Study the drawing (mm; zero at the part's minimum x, y, z) and answer. A direction names the side the tool comes from. Coordinates: 2 decimals unless noted, no trailing zeros. Write each loop counter-clockwise with the first axis right and the second up, starting at its lowest first coordinate (ties: lowest second). Pieces come first, ordered by that corner, then holes. Notation, with made-up numbers: (9, 24.5) - (60, 24.5) arc R13 ccw to (60, 47.5) - close; hole circle Ø10 at (1.25, 40). An arc over 180 degrees is marked (long way). One line per item, written item: value.
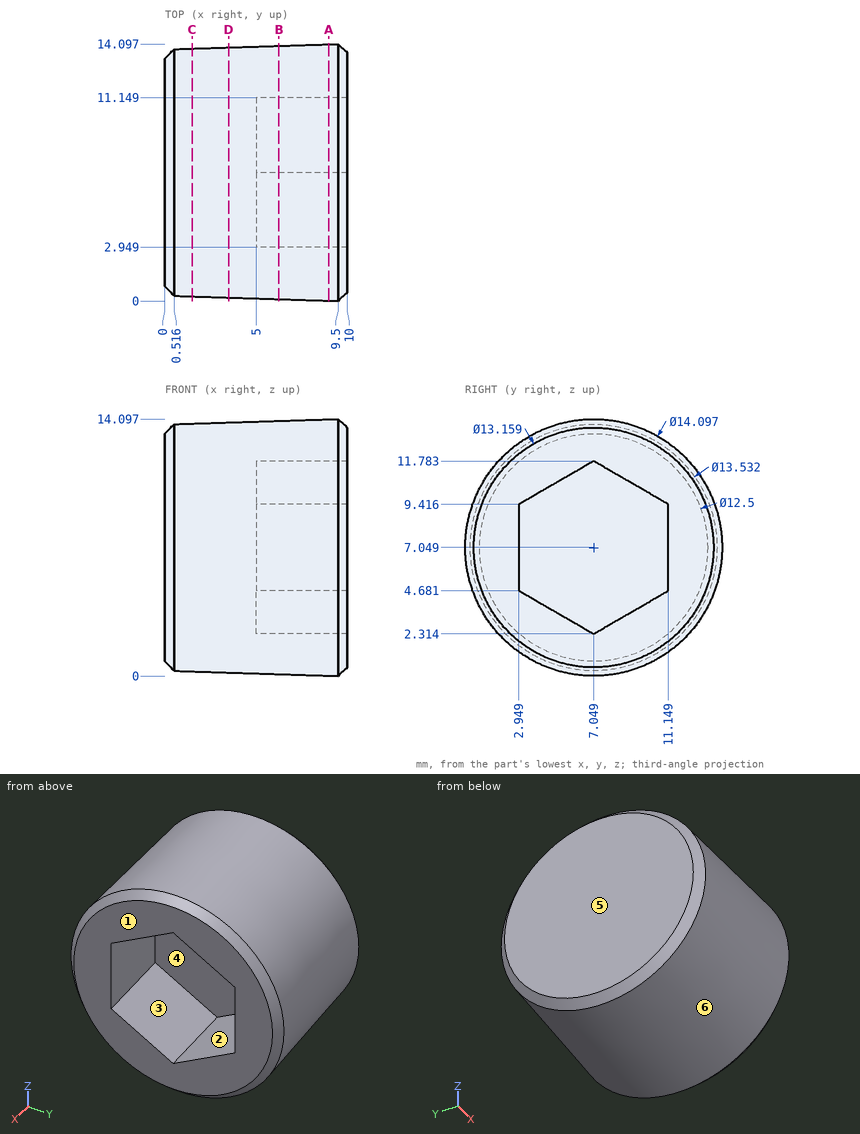
Item 1: Determine the mould class of the marked faces 3, 4, 5 and 6 for opening direction Y: +Y half, -Y half, draft (parallel to the pull), parting line (faces both ways), or undercut.
Evaluation:
face 3: undercut
face 4: undercut
face 5: draft
face 6: parting line
Item 2: Section C-C, the plane x = 1.5 is taken. Determine the outline of the cut face in (y, z) (1 decimal), then the cut area to 3 significant figures.
Evaluation:
outline: circle Ø13.6 at (7, 7)
area: 145 mm2
Item 3: Given pin 1 (6 mm diameter, centred on x = 2, z = 7, fed in from +Y); pin 2 (2 mm diameter, centred on y = 7, z = 4, fed in from -X); pin 3 (2.5 mm diameter, centred on y = 7, z = 7, fed in from +X); pin 4 (6 mm diameter, centred on x = 2, z = 12.5, fed in from -Y), each flat-ended and moving along its own axis, determine where each tip first touches the part or whether it passes through.
Evaluation:
pin 1: stops at y = 13.96
pin 2: stops at x = 0
pin 3: stops at x = 5
pin 4: stops at y = 0.69
Item 4: Section A-A, the plane x = 9 is taken. Determine the outline of the cut face in (y, z) (1 decimal).
Evaluation:
outline: circle Ø14.1 at (7, 7); hole (2.9, 4.7) - (7, 2.3) - (11.1, 4.7) - (11.1, 9.4) - (7, 11.8) - (2.9, 9.4) - close
Item 5: Section D-D, the plane x = 3.5 is taken. Determine the outline of the cut face in (y, z).
Evaluation:
outline: circle Ø13.72 at (7.05, 7.05)
Item 6: Which of the six approach directions +Z, -Z, +X, -X, +Y, -Y give full straight-line access (tool end or side, diameter ignored) to the marked faces 1 and 2?
Evaluation:
face 1: +Z, -Z, +X, +Y, -Y
face 2: +X
Item 7: Consider probe 1 along Z at (x, y) = (9, 5.5); probe 2 along X at (y, z) = (10, 9); probe 3 along Z at (x, y) = (6.25, 7) (1 decimal). Determine where each line is inside the solid, lowest interval first.
Evaluation:
probe 1: z = 0.19 to 3.21, 10.89 to 13.91
probe 2: x = 0 to 5
probe 3: z = 0.1 to 2.3, 11.8 to 14
Item 8: Section B-B, the plane x = 6.25 is taken. Determine the outline of the cut face in (y, z) (1 decimal).
Evaluation:
outline: circle Ø13.9 at (7, 7); hole (2.9, 4.7) - (7, 2.3) - (11.1, 4.7) - (11.1, 9.4) - (7, 11.8) - (2.9, 9.4) - close
